Read the model definition and answer for the solid it produces. Units are mm, in the model's axes. Face numbers are marked on the shaded views. A direction names the side the tool comes from. Round coordinates to 2 decimals unless told otherwise and drop trailing zeros. Write each loop counter-clockwise with the first axis right and the second up, starting at its lowest first coordinate (ties: lowest second). Pieces come first, ordered by that corner, then holes. Notation, with made-up numbers: (-32.5, -19) -> (13.5, -19) arc R23 cw to (13.5, 19) -> close; hole circle Ø6 at (-37, -6). An arc over 180 degrees is marked (long way). Return JSON: item names as keys, results as strings.
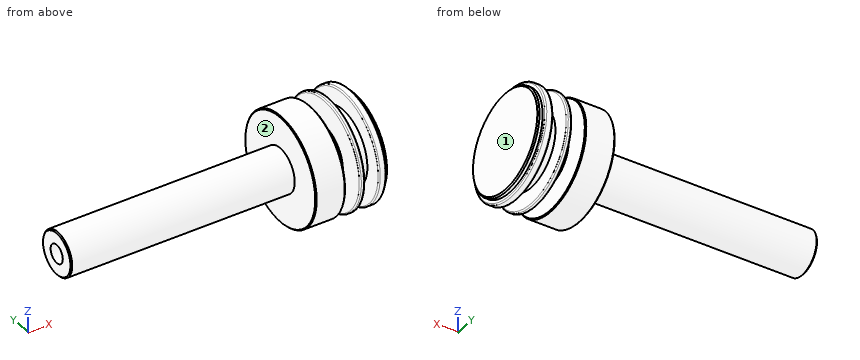
from build123d import *

# Parameters (mm, degrees)
M5_TAPPED_HOLE1_D     = 4.2
M5_TAPPED_HOLE1_DEPTH = 12.4
M5_TAPPED_HOLE1_TIP   = 1.2618073


with BuildPart() as part:
    # Sketch1 → Revolve1 (revolve)
    with BuildSketch(Plane.XY, mode=Mode.PRIVATE) as revolve1_sk:
        Polygon((-36, 0), (-36, 4.75), (-35.75, 5), (0, 5), (0, 0), align=None)
    revolve(revolve1_sk.sketch.rotate(Axis((0, 0, 0), (-1, 0, 0)), 270), axis=Axis((0, 0, 0), (-1, 0, 0)))

    # Sketch2 → Revolve2 (revolve)
    with BuildSketch(Plane.XY, mode=Mode.PRIVATE) as revolve2_sk:
        with BuildLine():
            Line((0, 0), (0, 5))
            Line((0, 5), (15, 5))
            Line((15, 5), (15, 12.1))
            Line((15, 12.1), (15.2, 12.3))
            Line((15.2, 12.3), (21.6, 12.3))
            Line((21.6, 12.3), (21.8, 12.1))
            Line((21.8, 12.1), (21.8, 6.5))
            Line((21.8, 6.5), (25, 6.5))
            Line((25, 6.5), (25, 12.15))
            ThreePointArc((25, 12.15), (25.087867966, 12.362132034), (25.3, 12.45))
            Line((25.3, 12.45), (25.8, 12.45))
            ThreePointArc((25.8, 12.45), (26.012132034, 12.362132034), (26.1, 12.15))
            Line((26.1, 12.15), (26.1, 8.45))
            Line((26.1, 8.45), (29.3, 8.45))
            Line((29.3, 8.45), (29.3, 12.15))
            ThreePointArc((29.3, 12.15), (29.387867966, 12.362132034), (29.6, 12.45))
            Line((29.6, 12.45), (30.7, 12.45))
            ThreePointArc((30.7, 12.45), (30.912132034, 12.362132034), (31, 12.15))
            Line((31, 12.15), (31, 11.45))
            Line((31, 11.45), (31.7, 11.45))
            Line((31.7, 11.45), (32, 11.15))
            Line((32, 11.15), (32, 0))
            Line((32, 0), (0, 0))
        make_face()
    revolve(revolve2_sk.sketch.rotate(Axis((32, 0, 0), (-1, 0, 0)), 270), axis=Axis((32, 0, 0), (-1, 0, 0)))

    # M5 Tapped Hole1
    with Locations(Plane.ZY.offset(36)):
        with Locations((0, 0)):
            Hole(M5_TAPPED_HOLE1_D / 2, depth=M5_TAPPED_HOLE1_DEPTH)
            with Locations((0, 0, -(M5_TAPPED_HOLE1_DEPTH + M5_TAPPED_HOLE1_TIP / 2))):  # 118° drill point
                Cone(0, M5_TAPPED_HOLE1_D / 2, M5_TAPPED_HOLE1_TIP, mode=Mode.SUBTRACT)


solid = part.part
Item 1: Flat-ended cylindrical pins translate along their axes: pin 1 (3 mm diameter, centred on x = 6, z = 0.5, fed in from -Y); pin 2 (2.5 mm diameter, centred on y = 0, z = 0, fed in from -X); pin 3 (12 mm diameter, centred on x = 6.5, z = -8, fed in from -Y). Find the tip coordinate at first contact, or state that the pin passes through.
Worked answers:
{"pin 1": "stops at y = -5", "pin 2": "stops at x = -23.09", "pin 3": "stops at y = -4.58"}
Item 2: Section A-A (x = 1.5) is taken. Give the vertices of the cut face in (y, z).
Worked answers:
{"outline": "circle Ø10 at (0, 0)"}
Item 3: Section B-B (z = 9.5) is taken. State how many separate pieces and enclosed holes the cut face has, then the cut area to 3 significant figures.
Worked answers:
{"separate pieces": "3", "enclosed holes": "0", "area": "164 mm2"}
Item 4: Straight lines are drawn through the part: L1, parallel to X at y = 3.5, z = 8.5; L2, parallel to X at y = -3, z = -6.25; L3, parallel to Y at x = -30.5, z = 0. For each, find the intervals that lie inside material, in ascending order. Write a range as [from, to].
Worked answers:
{"L1": "x = [15, 21.8], [25, 26.1], [29.3, 32]", "L2": "x = [15, 21.8], [25, 32]", "L3": "y = [-5, -2.1], [2.1, 5]"}
Item 5: A tool of negligible diameter and unlimited length cuts with its end or side. For the marked faces 1 and 2, from which of +Z, -Z, +X, -X, +Y, -Y can it reach the whole face along a straight path? Write none if from no direction.
Worked answers:
{"face 1": "+Z, -Z, +X, +Y, -Y", "face 2": "-X"}
Item 6: Section D-D (x = -26) is taken. Give the vertices of the cut face in (y, z).
Worked answers:
{"outline": "circle Ø10 at (0, 0); hole circle Ø4.2 at (0, 0)"}
